```python
from build123d import *

# Parameters (mm, degrees)
SKETCH1_R           = 15
SKETCH1_R_2         = 3
BOSS_EXTRUDE1_DEPTH = 5
CUT_EXTRUDE1_DEPTH  = 5
FILLET1_R           = 0.5


with BuildPart() as part:
    # Sketch1 → Boss-Extrude1 (new body)
    with BuildSketch(Plane.XY):
        Circle(SKETCH1_R)
        Circle(SKETCH1_R_2, mode=Mode.SUBTRACT)
    extrude(amount=BOSS_EXTRUDE1_DEPTH)

    # Sketch2 → Cut-Extrude1 (cut)
    with BuildSketch(Plane.XY.offset(5)):
        with BuildLine():
            Line((-5.153882032, 8.926785536), (-4.643543905, 8.042853971))
            ThreePointArc((-4.643543905, 8.042853971), (-3.630724563, 7.176652991), (-2.298547182, 7.13909524))
            ThreePointArc((-2.298547182, 7.13909524), (0, 7.5), (2.298547182, 7.13909524))
            ThreePointArc((2.298547182, 7.13909524), (3.630724563, 7.176652991), (4.643543905, 8.042853971))
            Line((4.643543905, 8.042853971), (5.153882032, 8.926785536))
            ThreePointArc((5.153882032, 8.926785536), (5.295294304, 10.626882735), (4.073608601, 11.817601828))
            ThreePointArc((4.073608601, 11.817601828), (0, 12.5), (-4.073608601, 11.817601828))
            ThreePointArc((-4.073608601, 11.817601828), (-5.295294304, 10.626882735), (-5.153882032, 8.926785536))
        make_face()
        with BuildLine():
            Line((8.926785536, 5.153882032), (8.042853971, 4.643543905))
            ThreePointArc((8.042853971, 4.643543905), (7.176652991, 3.630724563), (7.13909524, 2.298547182))
            ThreePointArc((7.13909524, 2.298547182), (7.5, 0), (7.13909524, -2.298547182))
            ThreePointArc((7.13909524, -2.298547182), (7.176652991, -3.630724563), (8.042853971, -4.643543905))
            Line((8.042853971, -4.643543905), (8.926785536, -5.153882032))
            ThreePointArc((8.926785536, -5.153882032), (10.626882735, -5.295294304), (11.817601828, -4.073608601))
            ThreePointArc((11.817601828, -4.073608601), (12.5, 0), (11.817601828, 4.073608601))
            ThreePointArc((11.817601828, 4.073608601), (10.626882735, 5.295294304), (8.926785536, 5.153882032))
        make_face()
        with BuildLine():
            Line((5.153882032, -8.926785536), (4.643543905, -8.042853971))
            ThreePointArc((4.643543905, -8.042853971), (3.630724563, -7.176652991), (2.298547182, -7.13909524))
            ThreePointArc((2.298547182, -7.13909524), (0, -7.5), (-2.298547182, -7.13909524))
            ThreePointArc((-2.298547182, -7.13909524), (-3.630724563, -7.176652991), (-4.643543905, -8.042853971))
            Line((-4.643543905, -8.042853971), (-5.153882032, -8.926785536))
            ThreePointArc((-5.153882032, -8.926785536), (-5.295294304, -10.626882735), (-4.073608601, -11.817601828))
            ThreePointArc((-4.073608601, -11.817601828), (0, -12.5), (4.073608601, -11.817601828))
            ThreePointArc((4.073608601, -11.817601828), (5.295294304, -10.626882735), (5.153882032, -8.926785536))
        make_face()
        with BuildLine():
            Line((-8.926785536, -5.153882032), (-8.042853971, -4.643543905))
            ThreePointArc((-8.042853971, -4.643543905), (-7.176652991, -3.630724563), (-7.13909524, -2.298547182))
            ThreePointArc((-7.13909524, -2.298547182), (-7.5, 0), (-7.13909524, 2.298547182))
            ThreePointArc((-7.13909524, 2.298547182), (-7.176652991, 3.630724563), (-8.042853971, 4.643543905))
            Line((-8.042853971, 4.643543905), (-8.926785536, 5.153882032))
            ThreePointArc((-8.926785536, 5.153882032), (-10.626882735, 5.295294304), (-11.817601828, 4.073608601))
            ThreePointArc((-11.817601828, 4.073608601), (-12.5, 0), (-11.817601828, -4.073608601))
            ThreePointArc((-11.817601828, -4.073608601), (-10.626882735, -5.295294304), (-8.926785536, -5.153882032))
        make_face()
    extrude(amount=-CUT_EXTRUDE1_DEPTH, mode=Mode.SUBTRACT)

    # Fillet1
    fillet1_edges = [part.edges().sort_by_distance(p)[0] for p in [
        (-15, 0, 0),
        (-15, 0, 5),
    ]]
    fillet(fillet1_edges, radius=FILLET1_R)


solid = part.part
```
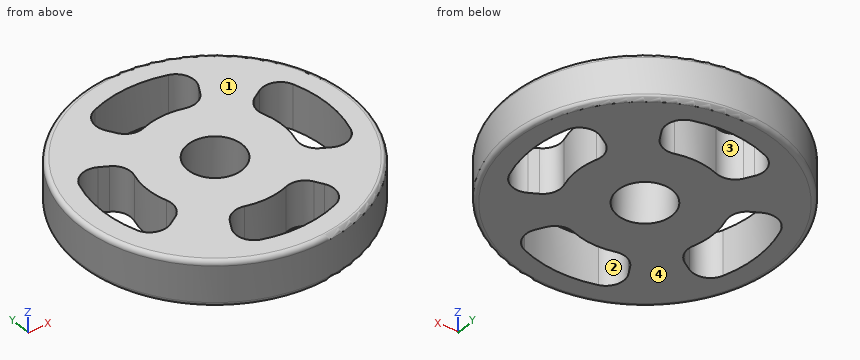
For this review, take the finished solid that the model builds, in its own axes (mm). Face numbers are marked on the shaded views. A direction names the side the tool comes from. Coordinates: 2 decimals unless noted, no trailing zeros. Order: outer loops, then holes, each group sorted by start corner. A loop starts at its lowest first (then second) coordinate and runs counter-clockwise, first axis right, second up. Notation, with made-up numbers: (37, 65.5) - (60, 65.5) arc R21 ccw to (60, 90.5) - close; hole circle Ø7 at (-25, -18). An arc over 180 degrees is marked (long way). Answer as a JSON object with one key per item and string values. Group by question number.
1. The part is to be moulded in two halves that separate along Y. For the marked faces 3 and 4, say which applies: pulls with the +Y half, pulls with the -Y half, needs draft (parallel to the pull), parting line crosses it, or undercut.
2. For probe 1 along Y at (x, z) = (0, 3.8); probe 2 along Y at (x, z) = (5, 1.55); probe 3 along X at (y, z) = (-0.5, 1.4), list the stretches that pass through material, from the lowest coordinate up.
3. Clearance check with flat-ended pins moving along their axes: P1, Ø1.5, axis at y = 12, z = 2.5, coming from the +X side; P2, Ø1.5, axis at x = -7.5, z = 3.5, coming from the -Y side; P3, Ø1, axis at y = 10, z = 3, coming from the +X side; P4, Ø3.5, axis at x = 0, y = 0, coming from the -Z side. State where each tip first meets the part, or that it passes through.
4. We need section A-A on x = 0. State the section outline as (y, z) points, then the cut area to 3 significant figures.
5. For the marked faces 1 and 2, list the 3-axis set-ups (+Z, -Z, +X, -X, +Y, -Y) from which the entire face can be reached by the end or side of a thin tool; tool diameter is ignored.
6. We need section C-C on z = 4.05. Give the number of separate pieces and of enclosed holes in the cut face, then the cut area to 3 significant figures.
Final values:
{
 "1": {"face 3": "undercut", "face 4": "needs draft"},
 "2": {"probe 1": "-15 to -12.5, -7.5 to -3, 3 to 7.5, 12.5 to 15", "probe 2": "-14.14 to -11.16, -8.66 to 8.66, 11.16 to 14.14", "probe 3": "-14.99 to -12.49, -7.48 to -2.96, 2.96 to 7.48, 12.49 to 14.99"},
 "3": {"P1": "x = 9.92", "P2": "y = -13.4", "P3": "x = 11.61", "P4": "through"},
 "4": {"outline": "(-15, 0.5) arc R0.5 ccw to (-14.5, 0) - (-12.5, 0) - (-12.5, 5) - (-14.5, 5) arc R0.5 ccw to (-15, 4.5) - close; (-7.5, 0) - (-3, 0) - (-3, 5) - (-7.5, 5) - close; (3, 0) - (7.5, 0) - (7.5, 5) - (3, 5) - close; (12.5, 0) - (14.5, 0) arc R0.5 ccw to (15, 0.5) - (15, 4.5) arc R0.5 ccw to (14.5, 5) - (12.5, 5) - close", "area": "69.8 mm²"},
 "5": {"face 1": "+Z, +X, -X, +Y, -Y", "face 2": "+Z, -Z"},
 "6": {"separate pieces": "1", "enclosed holes": "5", "area": "483 mm²"}
}
